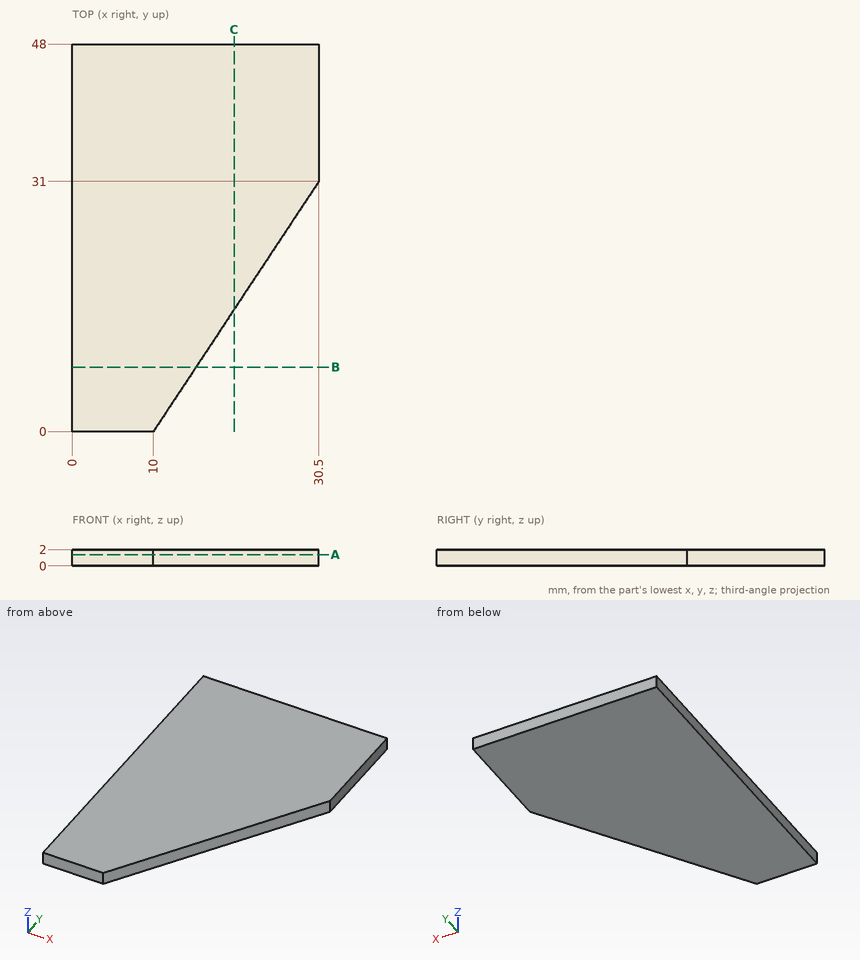
Check sheet for the drawn part. Datum: minimum x, y, z corner. Units: mm. Round coordinates to 2 decimals unless told otherwise and drop trailing zeros. Loops run counter-clockwise (first coordinate to the right, second up) from the corner with the lowest first, then second, coordinate; pieces in that order, holes last. Notation, with made-up numbers: (25, 31.25) - (84, 31.25) arc R25 ccw to (84, 46.25) - close; hole circle Ø1 at (19.5, 24). An arc over 180 degrees is marked (long way). Write each question's results on one line, items separated by ' | '. Start each with the question number.
Q1. Thickness scan on line 1 (X direction, y = 25, z = 1.1); line 2 (Y direction, x = 16.5, z = 0.8); line 3 (Y direction, x = 18, z = 0.8). Record the ranges inside material, lowest first. Write a range as [from, to].
Q2. Cross-section at C-C on x = 20. Enter the section's corners in (y, z).
Q3. Cross-section at B-B on y = 8. Enter the section's corners in (x, z).
Q4. Cross-section at A-A on z = 1.4. Enter the section's corners in (x, y).
Answers below:
1) line 1: x = [0, 26.53] | line 2: y = [9.83, 48] | line 3: y = [12.1, 48]
2) outline: (15.12, 0) - (48, 0) - (48, 2) - (15.12, 2) - close
3) outline: (0, 0) - (15.29, 0) - (15.29, 2) - (0, 2) - close
4) outline: (0, 0) - (10, 0) - (30.5, 31) - (30.5, 48) - (0, 48) - close
